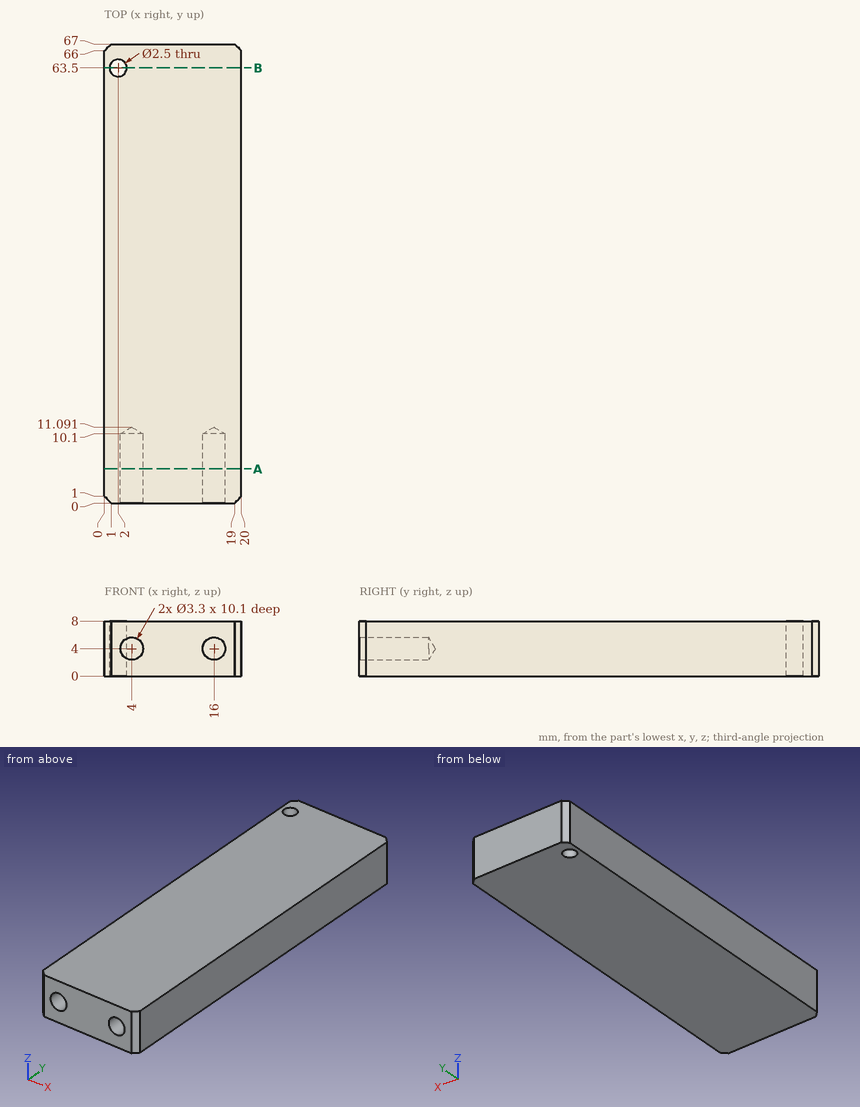
Could you check a few things on this drawing? It's one solid part, dimensions in mm from its lowest x, y, z. Round coordinates to 2 decimals unless told otherwise and drop trailing zeros. Loops run counter-clockwise (first coordinate to the right, second up) from the corner with the lowest first, then second, coordinate; pieces in that order, holes last.
Q1. I want a section at B-B (y = 63.5). Write out the boundary of the cut face in (x, z), and give its area (3 significant figures).
Q2. I want a section at A-A (y = 5). Write out the boundary of the cut face in (x, z).
Q3. Please list where these lines run through material, in increasing order: L1, parallel to X at y = 7.25, z = 4; L2, parallel to Y at x = 2, z = 2.25; L3, parallel to Z at x = 4, y = 4.25.
Answer below:
1. outline: (0, 0) - (0.75, 0) - (0.75, 8) - (0, 8) - close; (3.25, 0) - (20, 0) - (20, 8) - (3.25, 8) - close
1. area: 140 mm2
2. outline: (0, 0) - (20, 0) - (20, 8) - (0, 8) - close; hole circle Ø3.3 at (4, 4); hole circle Ø3.3 at (16, 4)
3. L1: x = 0 to 2.35, 5.65 to 14.35, 17.65 to 20
3. L2: y = 0 to 62.25, 64.75 to 67
3. L3: z = 0 to 2.35, 5.65 to 8
